Work out the finished part from the listing and answer in its coordinate system (mm). Face numbers are marked on the shaded views. A direction names the side the tool comes from. Give positions to 0.01 mm unless a question says otherwise; leave off trailing zeros. Order: outer loops, then holes, each group sorted by start corner. A loop starts at its lowest first (then second) coordinate and runs counter-clockwise, first axis right, second up. Notation, with made-up numbers: (1.5, 52.5) - (13.5, 52.5) arc R8 cw to (13.5, 56.5) - close; hole circle Ø8 at (43, -23.5). An arc over 180 degrees is marked (long way). Write each question's results on one line, items separated by ' | '.
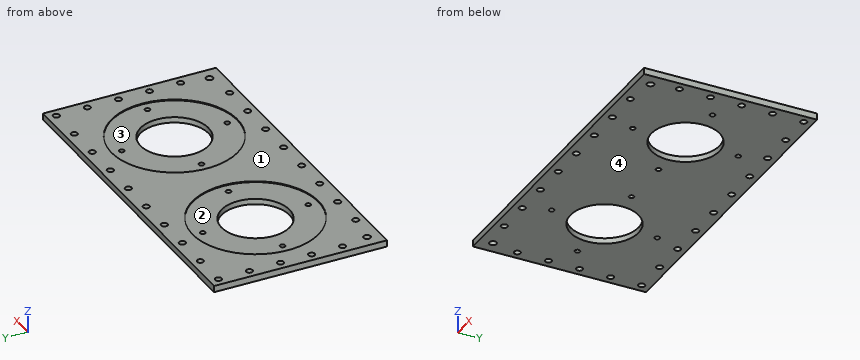
from build123d import *

# Parameters (mm, degrees)
SKETCH1_W           = 1140
SKETCH1_H           = 590
BOSS_EXTRUDE1_DEPTH = 22
SKETCH2_R           = 11
SKETCH2_R_2         = 12
CUT_EXTRUDE1_DEPTH  = 32
SKETCH3_R           = 116
CUT_EXTRUDE2_DEPTH  = 32
SKETCH4_R           = 215
CUT_EXTRUDE3_DEPTH  = 3
CIRPATTERN1_COUNT   = 4
CIRCPATTERN2_COUNT  = 4


with BuildPart() as part:
    # Sketch1 → Boss-Extrude1 (new body)
    with BuildSketch(Plane.XY):
        with Locations((138.473053892, -23.233532934)):
            Rectangle(SKETCH1_W, SKETCH1_H)
    extrude(amount=BOSS_EXTRUDE1_DEPTH)

    # Sketch2 → Cut-Extrude1 (cut)
    with BuildSketch(Plane.XY.offset(22)):
        with Locations((-401.526946108, 241.766467066)):
            Circle(SKETCH2_R)
        with Locations((-281.526946108, 241.766467066)):
            Circle(SKETCH2_R)
        with Locations((-161.526946108, 241.766467066)):
            Circle(SKETCH2_R)
        with Locations((-41.526946108, 241.766467066)):
            Circle(SKETCH2_R)
        with Locations((78.473053892, 241.766467066)):
            Circle(SKETCH2_R)
        with Locations((198.473053892, 241.766467066)):
            Circle(SKETCH2_R)
        with Locations((318.473053892, 241.766467066)):
            Circle(SKETCH2_R)
        with Locations((438.473053892, 241.766467066)):
            Circle(SKETCH2_R)
        with Locations((558.473053892, 241.766467066)):
            Circle(SKETCH2_R)
        with Locations((678.473053892, 241.766467066)):
            Circle(SKETCH2_R)
        with Locations((-386.526946108, -273.233532934)):
            Circle(SKETCH2_R_2)
        with Locations((558.473053892, -288.233532934)):
            Circle(SKETCH2_R)
        with Locations((438.473053892, -288.233532934)):
            Circle(SKETCH2_R)
        with Locations((318.473053892, -288.233532934)):
            Circle(SKETCH2_R)
        with Locations((198.473053892, -288.233532934)):
            Circle(SKETCH2_R)
        with Locations((78.473053892, -288.233532934)):
            Circle(SKETCH2_R)
        with Locations((-41.526946108, -288.233532934)):
            Circle(SKETCH2_R)
        with Locations((-161.526946108, -288.233532934)):
            Circle(SKETCH2_R)
        with Locations((-281.526946108, -288.233532934)):
            Circle(SKETCH2_R)
        with Locations((663.473053892, -273.233532934)):
            Circle(SKETCH2_R_2)
        with Locations((-401.526946108, 135.766467066)):
            Circle(SKETCH2_R)
        with Locations((-401.526946108, 29.766467066)):
            Circle(SKETCH2_R)
        with Locations((-401.526946108, -76.233532934)):
            Circle(SKETCH2_R)
        with Locations((-401.526946108, -182.233532934)):
            Circle(SKETCH2_R)
        with Locations((678.473053892, -182.233532934)):
            Circle(SKETCH2_R)
        with Locations((678.473053892, -76.233532934)):
            Circle(SKETCH2_R)
        with Locations((678.473053892, 29.766467066)):
            Circle(SKETCH2_R)
        with Locations((678.473053892, 135.766467066)):
            Circle(SKETCH2_R)
    extrude(amount=-CUT_EXTRUDE1_DEPTH, mode=Mode.SUBTRACT)

    # Sketch3 → Cut-Extrude2 (cut)
    with BuildSketch(Plane.XY.offset(22)):
        with Locations((-131.526946108, -23.233532934)):
            Circle(SKETCH3_R)
        with Locations((408.473053892, -23.233532934)):
            Circle(SKETCH3_R)
    extrude(amount=-CUT_EXTRUDE2_DEPTH, mode=Mode.SUBTRACT)

    # Sketch4 → Cut-Extrude3 (cut)
    with BuildSketch(Plane.XY.offset(22)):
        with Locations((-131.526946108, -23.233532934)):
            Circle(SKETCH4_R)
        with Locations((408.473053892, -23.233532934)):
            Circle(SKETCH4_R)
    extrude(amount=-CUT_EXTRUDE3_DEPTH, mode=Mode.SUBTRACT)

    # Sketch6 → M20 Tapped Hole1 (revolve, cut)
    with BuildSketch(Plane(origin=(-131.526946108, 156.766467066, 19), x_dir=(0, -1, 0), z_dir=(1, 0, 0))):
        Polygon((0, 0), (0, 57.757530416), (8.75, 52.5), (8.75, 0), align=None)
    m20_tapped_hole1 = revolve(axis=Axis((-131.526946108, 156.766467066, 25.35), (0, 0, -1)), mode=Mode.SUBTRACT)

    # CirPattern1: M20 Tapped Hole1 ×4 about axis
    cirpattern1_axis = Axis((-131.526946108, -23.233532934, 0), (0, 0, 1))
    for i in range(1, CIRPATTERN1_COUNT):
        add(m20_tapped_hole1.rotate(cirpattern1_axis, i * 360 / CIRPATTERN1_COUNT), mode=Mode.SUBTRACT)

    # Sketch8 → M20 Tapped Hole2 (revolve, cut)
    with BuildSketch(Plane(origin=(408.473053892, 156.766467066, 19), x_dir=(0, -1, 0), z_dir=(1, 0, 0))):
        Polygon((0, 0), (0, 57.757530416), (8.75, 52.5), (8.75, 0), align=None)
    m20_tapped_hole2 = revolve(axis=Axis((408.473053892, 156.766467066, 25.35), (0, 0, -1)), mode=Mode.SUBTRACT)

    # CircPattern2: M20 Tapped Hole2 ×4 about axis
    circpattern2_axis = Axis((408.473053892, -23.233532934, 0), (0, 0, 1))
    for i in range(1, CIRCPATTERN2_COUNT):
        add(m20_tapped_hole2.rotate(circpattern2_axis, i * 360 / CIRCPATTERN2_COUNT), mode=Mode.SUBTRACT)


solid = part.part
1. A tool of negligible diameter and unlimited length cuts with its end or side. For the marked faces 3 and 4, from which of +Z, -Z, +X, -X, +Y, -Y can it reach the whole face along a straight path? Write none if from no direction.
Answer list:
face 3: +Z | face 4: -Z, +X, -X, +Y, -Y
2. A cutting plane is placed at B-B, the plane x = 481. Write down the section's boundary in (y, z), then the cut area to 3 significant figures.
Answer list:
outline: (-318.23, 0) - (-113.76, 0) - (-113.76, 19) - (-225.63, 19) - (-225.63, 22) - (-318.23, 22) - close; (67.3, 0) - (271.77, 0) - (271.77, 22) - (179.16, 22) - (179.16, 19) - (67.3, 19) - close | area: 8,330 mm^2
3. Determine the mould class of the marked faces 1 and 2 for opening direction Y: +Y half, -Y half, draft (parallel to the pull), parting line (faces both ways), or undercut.
Answer list:
face 1: draft | face 2: undercut
4. A cutting plane is placed at D-D, the plane x = 348.5. Write down the section's boundary in (y, z).
Answer list:
outline: (-318.23, 0) - (-122.53, 0) - (-122.53, 19) - (-229.7, 19) - (-229.7, 22) - (-318.23, 22) - close; (76.06, 0) - (271.77, 0) - (271.77, 22) - (183.23, 22) - (183.23, 19) - (76.06, 19) - close
5. Straight lines are drawn through the part: line 1 (X direction, y = 117, z = 20.75); line 2 (X direction, y = 174, z = 19.5); line 3 (X direction, y = 29, z = 17.5). For each, find the intervals that lie inside material, in ascending order. Write a range as [from, to].
Answer list:
line 1: [-431.53, -294.5], [31.44, 245.5], [571.44, 708.47] | line 2: [-431.53, -217.11], [-45.95, 322.89], [494.05, 708.47] | line 3: [-431.53, -412.5], [-390.55, -235.1], [-27.95, 304.9], [512.05, 667.5], [689.45, 708.47]
6. A cutting plane is placed at C-C, the plane z = 4.75. State how many separate pieces and enclosed holes the cut face has, then the cut area to 3 significant figures.
Answer list:
separate pieces: 1 | enclosed holes: 38 | area: 575,000 mm^2
7. A cutting plane is placed at A-A, the plane y = 61.5. Write down the section's boundary in (x, z), then the cut area to 3 significant figures.
Answer list:
outline: (-431.53, 0) - (-210.75, 0) - (-210.75, 19) - (-329.13, 19) - (-329.13, 22) - (-431.53, 22) - close; (-52.3, 0) - (329.25, 0) - (329.25, 19) - (210.87, 19) - (210.87, 22) - (66.07, 22) - (66.07, 19) - (-52.3, 19) - close; (487.7, 0) - (708.47, 0) - (708.47, 22) - (606.07, 22) - (606.07, 19) - (487.7, 19) - close | area: 16,700 mm^2
